Here's the drawing with two shaded views (mm, measured from the low corner). I have some questions. A direction names the side the tool comes from. Round coordinates to 2 decimals unless told otherwise and drop trailing zeros. Loops run counter-clockwise (first coordinate to the right, second up) from the corner with the lowest first, then second, coordinate; pieces in that order, holes last. Notation, with made-up numbers: (47, -17.75) -> (77, -17.75) arc R8 ccw to (77, -2.75) -> close; hole circle Ø9 at (-36, 76.5). An arc over 180 degrees is marked (long way). Write each question's results on one line, items separated by ' | '.
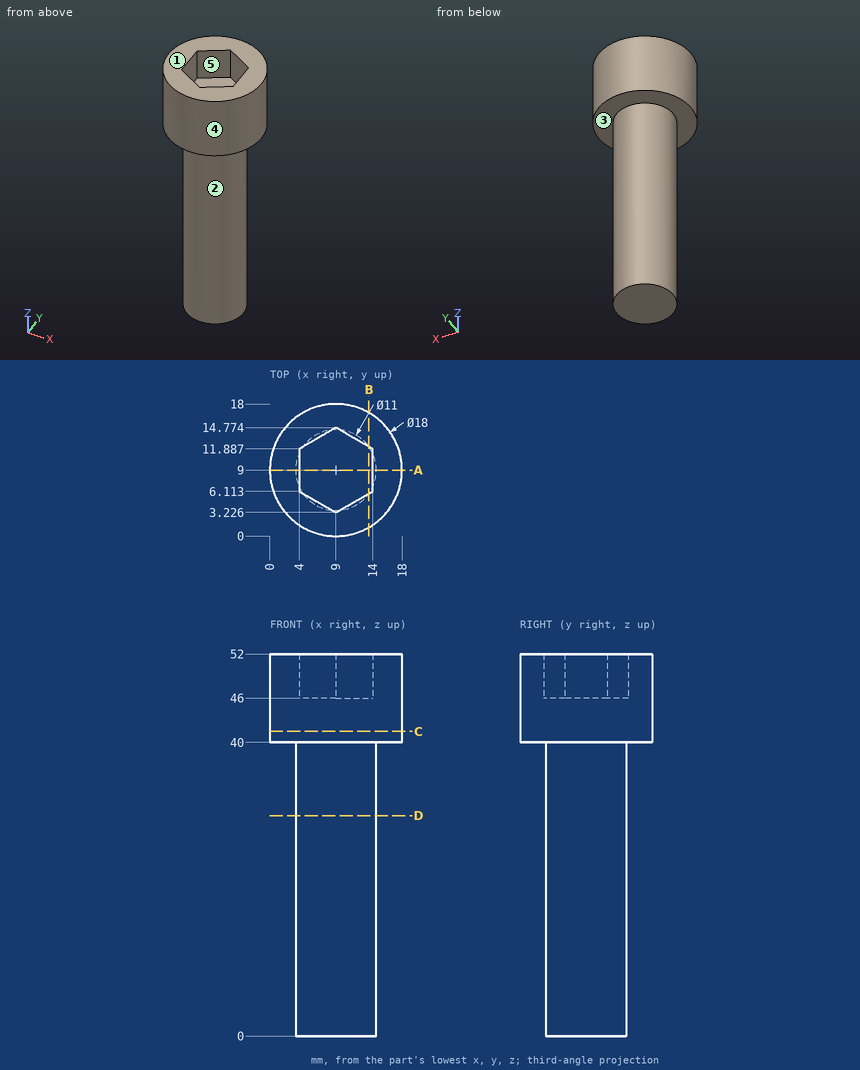
1. If we section it at B-B (x = 13.5): List the corners of the cut face in (y, z) for me (1 decimal).
Final values:
outline: (1.2, 40) -> (5.8, 40) -> (5.8, 0) -> (12.2, 0) -> (12.2, 40) -> (16.8, 40) -> (16.8, 52) -> (12.2, 52) -> (12.2, 46) -> (5.8, 46) -> (5.8, 52) -> (1.2, 52) -> close
2. We'd pull the mould along Y, two halves only. Please class the marked faces 3, 4 and 5: pulls with the +Y half, pulls with the -Y half, needs draft (parallel to the pull), parting line crosses it, or undercut.
Final values:
face 3: needs draft | face 4: parting line crosses it | face 5: undercut
3. If we section it at D-D (z = 30): List the corners of the cut face in (x, y) for me.
Final values:
outline: circle Ø11 at (9, 9)
4. Please list where these lines run through material, in increasing order: line 1 (Z direction, x = 6.5, y = 11.25); line 2 (Z direction, x = 6.75, y = 1.75); line 3 (Y direction, x = 9.25, z = 41). Write a range as from..to.
Final values:
line 1: 0..46 | line 2: 40..52 | line 3: 0..18
5. Will these pins go through, and if not, where does the flat tip stop? pin 1 (1.5 mm diameter, centred on x = 13.5, z = 18.5, fed in from +Y) (1 decimal); pin 2 (5.5 mm diameter, centred on x = 9.5, y = 11.5, fed in from -Z); pin 3 (6 mm diameter, centred on y = 16, z = 19, fed in from -X) (1 decimal); pin 4 (1 mm diameter, centred on x = 11, z = 13.5, fed in from -Y).
Final values:
pin 1: y = 13 | pin 2: z = 0 | pin 3: x = 5.2 | pin 4: y = 3.71
6. If we section it at C-C (z = 41.5): List the corners of the cut face in (x, y) for me.
Final values:
outline: circle Ø18 at (9, 9)
7. On a 3-axis mill with a long thin cutter (end or side, diameter ignored), from which of +Z, -Z, +X, -X, +Y, -Y can I reach the whole of each face in a straight line? I mean the marked faces 1 and 2. Say none if no direction works.
Final values:
face 1: +Z, +X, -X, +Y, -Y | face 2: -Z
8. If we section it at A-A (y = 9): List the corners of the cut face in (x, z) for me, then the cut area to 3 significant figures.
Final values:
outline: (0, 40) -> (3.5, 40) -> (3.5, 0) -> (14.5, 0) -> (14.5, 40) -> (18, 40) -> (18, 52) -> (14, 52) -> (14, 46) -> (4, 46) -> (4, 52) -> (0, 52) -> close | area: 596 mm2
